```python
from build123d import *

# Parameters (mm, degrees)
SKETCH1_R               = 485
SKETCH1_R_2             = 465
BOSS_EXTRUDE1_DEPTH     = 700
CUT_EXTRUDE1_DEPTH      = 981.025509872
CUT_EXTRUDE1_DEPTH_BACK = 981.025509872
SKETCH2_W               = 247.5
SKETCH2_H               = 300
SKETCH3_R               = 17.5
CUT_EXTRUDE2_DEPTH      = 700


with BuildPart() as part:
    # Sketch1 → Boss-Extrude1 (new body)
    with BuildSketch(Plane.XY):
        Circle(SKETCH1_R)
        Circle(SKETCH1_R_2, mode=Mode.SUBTRACT)
    extrude(amount=BOSS_EXTRUDE1_DEPTH)

    # Sketch2 → Cut-Extrude1 (cut, two sides: drawn at the far end of the back side and taken through both)
    with BuildSketch(Plane(origin=(0, 0, 0), x_dir=(1, 0, 0), z_dir=(0, 1, 0)).offset(-CUT_EXTRUDE1_DEPTH_BACK)):
        with Locations((361.25, -350)):
            Rectangle(SKETCH2_W, SKETCH2_H)
        with Locations((-361.25, -350)):
            Rectangle(SKETCH2_W, SKETCH2_H)
    extrude(amount=CUT_EXTRUDE1_DEPTH + CUT_EXTRUDE1_DEPTH_BACK, mode=Mode.SUBTRACT)

    # Sketch3 → Cut-Extrude2 (cut)
    with BuildSketch(Plane(origin=(0, 0, 0), x_dir=(1, 0, 0), z_dir=(0, 1, 0))):
        with Locations(Location((180, -220, 0), (0, 0, 90))):
            Circle(SKETCH3_R)
        with Locations(Location((180, -480, 0), (0, 0, 90))):
            Circle(SKETCH3_R)
    extrude(amount=CUT_EXTRUDE2_DEPTH, mode=Mode.SUBTRACT)


solid = part.part
```
The listing builds one solid part. Answer for the finished solid, in the listing's coordinates (mm). A direction names the side the tool comes from. Coordinates: 2 decimals unless noted, no trailing zeros. Loops run counter-clockwise (first coordinate to the right, second up) from the corner with the lowest first, then second, coordinate; pieces in that order, holes last. Notation, with made-up numbers: M -16,23 L -9,23 A19 ccw -9,37 Z; hole C -7.75,54.5 d5. An arc over 180 degrees is marked long. Answer as CSV lines item,"result". Start each with the question number.
(1) For faces 4 (the cylindrical face through (186.703, 438.72, 203.834)), 5 (the flat face through (393, -249, 700)), determine the directions among +Z, -Z, +X, -X, +Y, -Y from which every point of the face is accessible in a straight line to the end or side of a thin tool.
(2) Given pin 1 (3 mm diameter, centred on x = -87, z = 476, fed in from -Y); pin 2 (7 mm diameter, centred on y = -408.5, z = 361.5, fed in from -X); pin 3 (7 mm diameter, centred on y = 410.5, z = 357, fed in from +X), each flat-ended and moving along its own axis, determine where each tip first touches the part or whether it passes through.
(3) The mould has two halves that part along Y. Classify faces 1 (the cylindrical face through (186.703, 438.72, 463.834)), 2 (the cylindrical face through (223.798, -430.278, 345.1)), 3 (the cylindrical face through (214.569, -412.535, 345.1)): pulls with the +Y half, pulls with the -Y half, needs draft (parallel to the pull), parting line crosses it, or undercut.
(4) The part is cut by section B-B (y = 0). Give the vertices of the cut face in (x, z), and give its area (3 significant figures).
(5) The part is cut by section A-A (z = 416). Give the vertices of the cut face in (x, y), and give its area (3 significant figures).
(6) The part is cut by section C-C (x = 0). Give the vertices of the cut face in (y, z), and give its area (3 significant figures).
(7) Find the intervals of material crossed by L1, parallel to Z at x = 180, y = 431; L2, parallel to Y at x = 0, z = 310; L3, parallel to Y at x = 141.5, z = 302, in increasing order. Write a range as [from, to].
(8) The part is cut by section D-D (x = -319.5). Give the vertices of the cut face in (y, z).
Determined:
1,face 4,"+Y"
1,face 5,"+Z, +X, -X, +Y, -Y"
2,pin 1,"y = -477.4"
2,pin 2,"x = -237.5"
2,pin 3,"x = 237.5"
3,face 1,"needs draft"
3,face 2,"parting line crosses it"
3,face 3,"undercut"
4,outline,"M -485,0 L -465,0 L -465,200 L -485,200 Z; M -485,500 L -465,500 L -465,700 L -485,700 Z; M 465,0 L 485,0 L 485,200 L 465,200 Z; M 465,500 L 485,500 L 485,700 L 465,700 Z"
4,area,"16,000 mm2"
5,outline,"M -237.5,-422.87 A485 ccw 237.5,-422.87 L 237.5,-399.77 A465 cw -237.5,-399.77 Z; M -237.5,399.77 A465 cw 237.5,399.77 L 237.5,422.87 A485 ccw -237.5,422.87 Z"
5,area,"19,900 mm2"
6,outline,"M -485,0 L -465,0 L -465,700 L -485,700 Z; M 465,0 L 485,0 L 485,700 L 465,700 Z"
6,area,"28,000 mm2"
7,L1,"[0, 202.5], [237.5, 462.5], [497.5, 700]"
7,L2,"[-485, -465], [465, 485]"
7,L3,"[-463.9, -442.95], [442.95, 463.9]"
8,outline,"M -364.89,0 L -337.85,0 L -337.85,200 L -364.89,200 Z; M -364.89,500 L -337.85,500 L -337.85,700 L -364.89,700 Z; M 337.85,0 L 364.89,0 L 364.89,200 L 337.85,200 Z; M 337.85,500 L 364.89,500 L 364.89,700 L 337.85,700 Z"
